Input: dimensioned drawing with shaded views. Units: mm. Origin: part minimum x, y, z. Round coordinates to 2 decimals unless told otherwise and drop trailing zeros. Loops run counter-clockwise (first coordinate to the right, second up) from the corner with the lowest first, then second, coordinate; pieces in that order, holes last. Notation, with made-up numbers: M 56,84.25 L 111,84.25 A15 ccw 111,100.25 Z; hole C 63.5,73 d2. An arc over 180 degrees is marked long. Put each result on its own line as item: value. Start each with the question number.
1) Line query: probe 1 along Z at (x, y) = (88, 343); probe 2 along Z at (x, y) = (107, 507.5); probe 3 along X at (y, z) = (258, 288). Output: solid intervals per line, ascending.
2) Section C-C on z = 271. Output: boundary loops of the cut face in (x, y), plus the area to 3 significant figures.
3) Section B-B on y = 93. Output: boundary loops of the cut face in (x, z), plus the area to 4 significant figures.
4) Section A-A on x = 100. Output: boundary loops of the cut face in (y, z).
5) Pin query (flat end, axial travel): pin 1 (12 mm diameter, centred on y = 331, z = 263, fed in from +X); pin 2 (6 mm diameter, centred on x = 92.5, y = 520.5, fed in from +Z). Return the tip coordinate at first contact, or that it passes through.
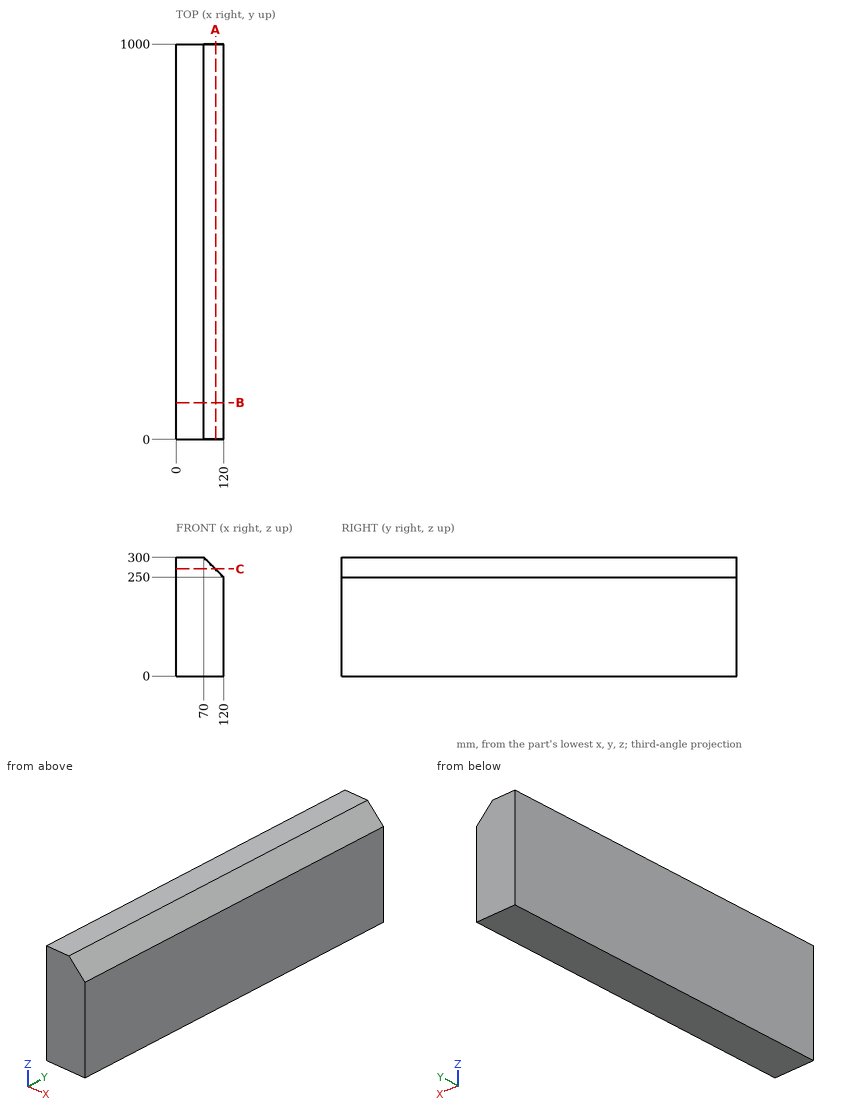
Geometry results:
1. probe 1: z = 0 to 282
1. probe 2: z = 0 to 263
1. probe 3: x = 0 to 82
2. outline: M 0,0 L 99,0 L 99,1000 L 0,1000 Z
2. area: 99,000 mm²
3. outline: M 0,0 L 120,0 L 120,250 L 70,300 L 0,300 Z
3. area: 34,750 mm²
4. outline: M 0,0 L 1000,0 L 1000,270 L 0,270 Z
5. pin 1: stops at x = 113
5. pin 2: stops at z = 280.5
